For this review, take the finished solid that the model builds, in its own axes (mm). A direction names the side the tool comes from. Coordinates: 2 decimals unless noted, no trailing zeros. Loops run counter-clockwise (first coordinate to the right, second up) from the corner with the lowest first, then second, coordinate; pieces in that order, holes last. Notation, with made-up numbers: (16, 61.5) -> (30, 61.5) arc R25 ccw to (30, 76.5) -> close; hole circle Ø6 at (68.25, -16.5). An arc over 180 degrees is marked (long way). Use a Markdown table: item, result.
from build123d import *

# Parameters (mm, degrees)
SKETCH1_W                                           = 200
SKETCH1_H                                           = 200
BOSS_EXTRUDE1_DEPTH                                 = 5
SKETCH2_R                                           = 7.5
CUT_EXTRUDE1_DEPTH                                  = 10
LPATTERN1_COUNT                                     = 2
LPATTERN1_PITCH                                     = 180
LPATTERN1_COUNT_DIR2                                = 3
LPATTERN1_PITCH_DIR2                                = 80
HOLE_SIZE_BASED_ON_SOCKET_HEAD_CAP_SCRE_D           = 6.6
HOLE_SIZE_BASED_ON_SOCKET_HEAD_CAP_SCRE_CBORE_D     = 11
HOLE_SIZE_BASED_ON_SOCKET_HEAD_CAP_SCRE_CBORE_DEPTH = 6.8


with BuildPart() as part:
    # Sketch1 → Boss-Extrude1 (new, symmetric)
    with BuildSketch(Plane(origin=(0, 0, 0), x_dir=(1, 0, 0), z_dir=(0, 1, 0))):
        Rectangle(SKETCH1_W, SKETCH1_H)
    extrude(amount=BOSS_EXTRUDE1_DEPTH, both=True)

    # Sketch2 → Cut-Extrude1 (cut)
    with BuildSketch(Plane(origin=(0, 5, 0), x_dir=(1, 0, 0), z_dir=(0, 1, 0))):
        with Locations(Location((80, 90, 0), (0, 0, 270))):
            Circle(SKETCH2_R)
    cut_extrude1 = extrude(amount=-CUT_EXTRUDE1_DEPTH, mode=Mode.SUBTRACT)

    # LPattern1: Cut-Extrude1 2 × 3
    with Locations(*[(-j * LPATTERN1_PITCH_DIR2, 0, i * LPATTERN1_PITCH) for i in range(LPATTERN1_COUNT) for j in range(LPATTERN1_COUNT_DIR2) if (i, j) != (0, 0)]):
        add(cut_extrude1, mode=Mode.SUBTRACT)

    # Hole Size (based on socket head cap screw type)1 (through all)
    with Locations(Plane(origin=(0, 5, 0), x_dir=(1, 0, 0), z_dir=(0, 1, 0))):
        with Locations((25, 25), (25, -25), (-25, 25), (-25, -25)):
            CounterBoreHole(HOLE_SIZE_BASED_ON_SOCKET_HEAD_CAP_SCRE_D / 2, HOLE_SIZE_BASED_ON_SOCKET_HEAD_CAP_SCRE_CBORE_D / 2, HOLE_SIZE_BASED_ON_SOCKET_HEAD_CAP_SCRE_CBORE_DEPTH)


solid = part.part
(1) Take a section at C-C on y = 2.5. State how many separate pieces and enclosed holes the cut face has, plus the area to 3 significant figures.
Found:
| item | result |
|---|---|
| separate pieces | 1 |
| enclosed holes | 10 |
| area | 38,600 mm^2 |
(2) For line 1 along X through (y, z) = (-0.5, -90); line 2 along X through (y, z) = (3.25, 25); line 3 along Z through (x, y) = (26, -3), list the stretches that pass through material, from the lowest coordinate up.
Found:
| item | result |
|---|---|
| line 1 | x = -100 to -87.5, -72.5 to -7.5, 7.5 to 72.5, 87.5 to 100 |
| line 2 | x = -100 to -30.5, -19.5 to 19.5, 30.5 to 100 |
| line 3 | z = -100 to -28.14, -21.86 to 21.86, 28.14 to 100 |
(3) Take a section at D-D on x = -25. Write out the cut boundary in (y, z).
Found:
| item | result |
|---|---|
| outline | (-5, -100) -> (5, -100) -> (5, -30.5) -> (-1.8, -30.5) -> (-1.8, -28.3) -> (-5, -28.3) -> close; (-5, -21.7) -> (-1.8, -21.7) -> (-1.8, -19.5) -> (5, -19.5) -> (5, 19.5) -> (-1.8, 19.5) -> (-1.8, 21.7) -> (-5, 21.7) -> close; (-5, 28.3) -> (-1.8, 28.3) -> (-1.8, 30.5) -> (5, 30.5) -> (5, 100) -> (-5, 100) -> close |
(4) Mouldability with a two-part tool opening along Z and no side actions: class faces 1 (the face through (-1, 0, 100)), 2 (the face through (-19.754, 1.648, -26.652)), 3 (the face through (-1, -5, -1)) as pulls with the +Z half, pulls with the -Z half, needs draft (parallel to the pull), parting line crosses it, or undercut.
Found:
| item | result |
|---|---|
| face 1 | pulls with the +Z half |
| face 2 | undercut |
| face 3 | needs draft |
(5) Take a section at B-B on z = 25. Write out the cut boundary in (x, y).
Found:
| item | result |
|---|---|
| outline | (-100, -5) -> (-28.3, -5) -> (-28.3, -1.8) -> (-30.5, -1.8) -> (-30.5, 5) -> (-100, 5) -> close; (-21.7, -5) -> (21.7, -5) -> (21.7, -1.8) -> (19.5, -1.8) -> (19.5, 5) -> (-19.5, 5) -> (-19.5, -1.8) -> (-21.7, -1.8) -> close; (28.3, -5) -> (100, -5) -> (100, 5) -> (30.5, 5) -> (30.5, -1.8) -> (28.3, -1.8) -> close |
(6) Take a section at A-A on x = -80. Write out the cut boundary in (y, z).
Found:
| item | result |
|---|---|
| outline | (-5, -100) -> (5, -100) -> (5, -97.5) -> (-5, -97.5) -> close; (-5, -82.5) -> (5, -82.5) -> (5, 82.5) -> (-5, 82.5) -> close; (-5, 97.5) -> (5, 97.5) -> (5, 100) -> (-5, 100) -> close |
(7) For faces 4 (the face through (-28.05, -3.42, 26.26)), 5 (the face through (-25, -1.8, -21)), list the 3-axis set-ups (+Z, -Z, +X, -X, +Y, -Y) from which the entire face can be reached by the end or side of a thin tool; tool diameter is ignored.
Found:
| item | result |
|---|---|
| face 4 | +Y, -Y |
| face 5 | +Y |
(8) For pin 1 Ø8.5 at (x, z) = (25, 25) entering from +Y, flat-tipped, find the tip position at first contact; note if it passes through.
Found:
| item | result |
|---|---|
| pin 1 | stops at y = -1.8 |
